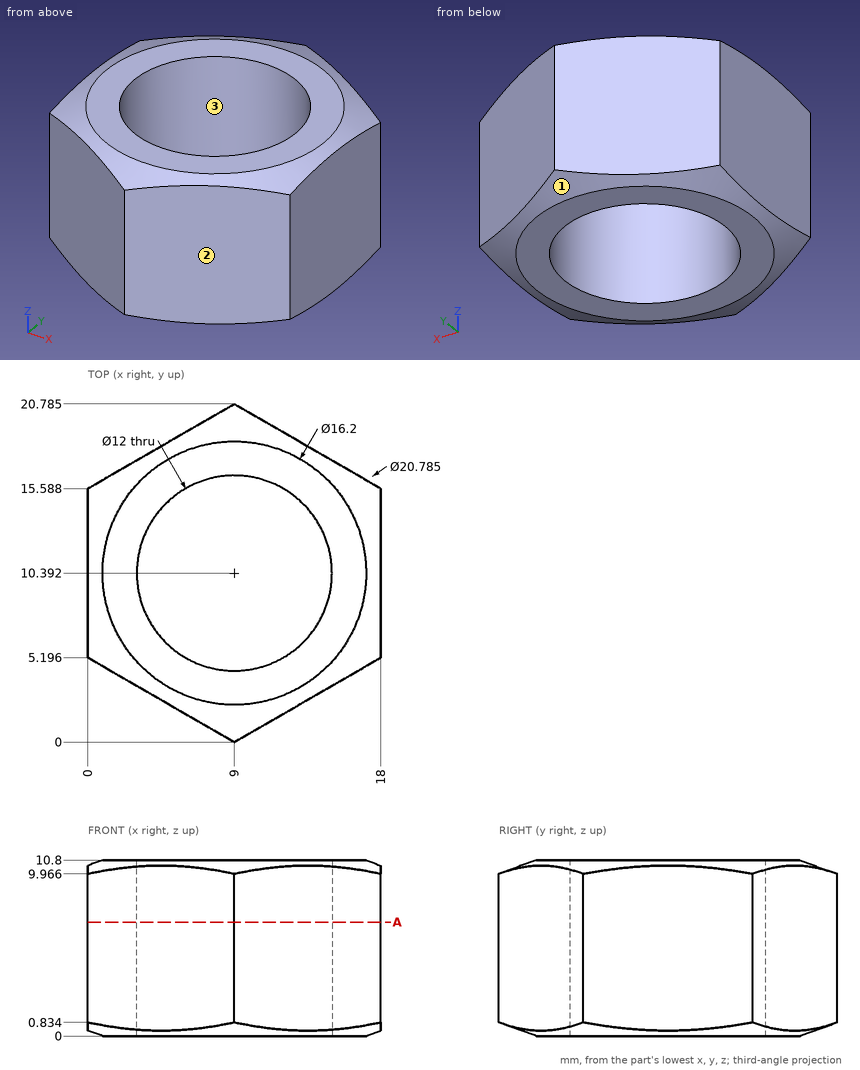
Verification items for this drawing (mm, ordinates from the low corner). Coordinates: 2 decimals unless noted, no trailing zeros. Write each loop counter-clockwise with the first axis right and the second up, starting at its lowest first coordinate (ties: lowest second). Pieces come first, ordered by that corner, then holes. Notation, with made-up numbers: M 45,-15.75 L 68,-15.75 A26 cw 68,-1.75 Z; hole C 11.5,85.5 d6. An arc over 180 degrees is marked long. Answer as a JSON object with one key per item and string values. Group by question number.
(1) Material ranges on line 1 (Y direction, x = 5, z = 4) (1 decimal); line 2 (Y direction, x = 9.25, z = 4.5) (1 decimal); line 3 (X direction, y = 5.5, z = 5.25) (1 decimal), recorded low to high.
(2) Gauge pin test, flat ends, axial feed: pin 1 (4 mm diameter, centred on x = 3, z = 4, fed in from -Y); pin 2 (4 mm diameter, centred on x = 8, z = 2, fed in from +Y) (1 decimal); pin 3 (2 mm diameter, centred on x = 2.5, z = 6.5, fed in from +Y). Record the tip position at first contact, or that the pin passes through.
(3) Cross-section at A-A, the plane z = 7. Record the cut outline in (x, y) (1 decimal).
(4) Release check for a two-part mould opening along Y. For the marked faces 1, 2 and 3 record: +Y half, -Y half, draft (parallel to the pull), parting line (faces both ways), or undercut.
Reply:
{
 "1": {"line 1": "2.3 to 5.9, 14.9 to 18.5", "line 2": "0.1 to 4.4, 16.4 to 20.6", "line 3": "0 to 5.5, 12.5 to 18"},
 "2": {"pin 1": "y = 2.31", "pin 2": "y = 20.8", "pin 3": "y = 17.61"},
 "3": {"outline": "M 0,5.2 L 9,0 L 18,5.2 L 18,15.6 L 9,20.8 L 0,15.6 Z; hole C 9,10.4 d12"},
 "4": {"face 1": "parting line", "face 2": "-Y half", "face 3": "undercut"}
}
